Geometry check sheet. Reference: the model listing, model coordinates, mm. A direction names the side the tool comes from. Give positions to 0.01 mm unless a question says otherwise; leave off trailing zeros. Order: outer loops, then holes, each group sorted by start corner. A loop starts at its lowest first (then second) coordinate and runs counter-clockwise, first axis right, second up.
```python
from build123d import *

# Parameters (mm, degrees)
SKETCH1_R                       = 5
BOSS_EXTRUDE1_DEPTH             = 60
SKETCH2_W                       = 20
SKETCH2_H                       = 20
CUT_EXTRUDE1_DEPTH              = 1.5
M5_TAPPED_HOLE1_D               = 4.2
M5_TAPPED_HOLE1_DEPTH           = 15
M5_TAPPED_HOLE1_TIP             = 1.2618073
M5_TAPPED_HOLE1_ON_FACE_2_D     = 4.2
M5_TAPPED_HOLE1_ON_FACE_2_DEPTH = 15
M5_TAPPED_HOLE1_ON_FACE_2_TIP   = 1.2618073


with BuildPart() as part:
    # Sketch1 → Boss-Extrude1 (new body)
    with BuildSketch(Plane.XY):
        with Locations((-90, 55)):
            Circle(SKETCH1_R)
    extrude(amount=BOSS_EXTRUDE1_DEPTH)

    # Sketch2 → Cut-Extrude1 (cut)
    with BuildSketch(Plane(origin=(0, 60, 0), x_dir=(1, 0, 0), z_dir=(0, 1, 0))):
        with Locations((-90, -30)):
            Rectangle(SKETCH2_W, SKETCH2_H)
    cut_extrude1 = extrude(amount=-CUT_EXTRUDE1_DEPTH, mode=Mode.SUBTRACT)

    # Mirror1: Cut-Extrude1 across plane
    add(cut_extrude1.mirror(Plane.ZX.offset(55)), mode=Mode.SUBTRACT)

    # M5 Tapped Hole1
    with Locations(Plane(origin=(-90, 55, 0), x_dir=(-1, 0, 0), z_dir=(0, 0, -1))):
        with Locations((0, 0)):
            Hole(M5_TAPPED_HOLE1_D / 2, depth=M5_TAPPED_HOLE1_DEPTH)
            with Locations((0, 0, -(M5_TAPPED_HOLE1_DEPTH + M5_TAPPED_HOLE1_TIP / 2))):  # 118° drill point
                Cone(0, M5_TAPPED_HOLE1_D / 2, M5_TAPPED_HOLE1_TIP, mode=Mode.SUBTRACT)

    # M5 Tapped Hole1 on face 2
    with Locations(Plane(origin=(-90, 55, 60), x_dir=(1, 0, 0), z_dir=(0, 0, 1))):
        with Locations((0, 0)):
            Hole(M5_TAPPED_HOLE1_ON_FACE_2_D / 2, depth=M5_TAPPED_HOLE1_ON_FACE_2_DEPTH)
            with Locations((0, 0, -(M5_TAPPED_HOLE1_ON_FACE_2_DEPTH + M5_TAPPED_HOLE1_ON_FACE_2_TIP / 2))):  # 118° drill point
                Cone(0, M5_TAPPED_HOLE1_ON_FACE_2_D / 2, M5_TAPPED_HOLE1_ON_FACE_2_TIP, mode=Mode.SUBTRACT)


solid = part.part
```
Q1. Release check for a two-part mould opening along Z. For faces 1 (the face through (-87.8, 54, 0)), 2 (the face through (-95, 55, 30)), 3 (the face through (-90, 59, 40)), 4 (the face through (-90.27, 55.25, 43.96)) record: pulls with the +Z half, pulls with the -Z half, needs draft (parallel to the pull), parting line crosses it, or undercut.
Q2. Cross-section at C-C, the plane z = 30. Record the boundary of the cut face in (x, y).
Q3. Cross-section at A-A, the plane x = -87. Record the boundary of the cut face in (y, z), and give its area (3 significant figures).
Q4. Gauge pin test, flat ends, axial feed: P1, Ø6, axis at x = -90.5, z = 33.5, coming from the +Y side; P2, Ø5.5, axis at x = -91.5, z = 31.5, coming from the -Y side; P3, Ø6, axis at x = -86.5, z = 19, coming from the -Y side. Record the tip position at first contact, or that the pin passes through.
Q5. Access from +Z, -Z, +X, -X, +Y, -Y to the whole of each face (thin tool, end or side, straight path). Record for faces 5 (the face through (-90, 51.5, 30)), 6 (the face through (-88.334, 53.722, 52.395)), 7 (the face through (-91.666, 53.722, 7.605)).
Q6. Thickness scan on L1, parallel to Y at x = -90, z = 7.25; L2, parallel to Z at x = -91.75, y = 59.25; L3, parallel to X at y = 51.5, z = 46. Record the ranges inside material, lowest first.
Q7. Cross-section at B-B, the plane y = 58. Record the boundary of the cut face in (x, z), and give its area (3 significant figures).
Answers follow:
1. face 1: pulls with the -Z half
1. face 2: needs draft
1. face 3: undercut
1. face 4: pulls with the +Z half
2. outline: (-93.57, 51.5) - (-86.43, 51.5) arc R5 ccw to (-86.43, 58.5) - (-93.57, 58.5) arc R5 ccw to start
3. outline: (51, 0) - (59, 0) - (59, 20) - (58.5, 20) - (58.5, 40) - (59, 40) - (59, 60) - (51, 60) - (51, 40) - (51.5, 40) - (51.5, 20) - (51, 20) - close
3. area: 460 mm2
4. P1: stops at y = 58.5
4. P2: stops at y = 51.5
4. P3: stops at y = 50.03
5. face 5: +X, -X, -Y
5. face 6: +Z
5. face 7: -Z
6. L1: y = 50 to 52.9, 57.1 to 60
6. L2: z = 0 to 20, 40 to 60
6. L3: x = -93.57 to -86.43
7. outline: (-94, 0) - (-86, 0) - (-86, 60) - (-94, 60) - close
7. area: 480 mm2
